Answer from the drawing. Dimensions are ordinates in mm from the lowest x, y and z of the part. A direction names the side the tool comes from. Give positions to 0.01 mm unless a question says otherwise; leave off trailing zeros. Loops run counter-clockwise (first coordinate to the right, second up) from the corner with the lowest first, then second, coordinate; pieces in that order, holes last.
Item 1: Section D-D, the plane x = 18 is taken. Give the vertices of the cut face in (y, z), and give its area (3 significant figures).
Item 2: Each of these flat-tipped pins is pushed along its axis until it touches: pin 1 Ø2 at (y, z) = (20.5, 26.5) entering from +X; pin 2 Ø10 at (x, y) = (26.5, 36) entering from +Z. Where does it stop, or does it pass through?
Item 3: A tool of negligible diameter and unlimited length cuts with its end or side. For the marked faces 1, 2 and 3, from which of +Z, -Z, +X, -X, +Y, -Y can it reach the whole face along a straight path? Write none if from no direction.
Item 4: Section B-B, the plane y = 41 is taken. Give the vertices of the cut face in (x, z).
Item 5: Consider line 1 along Y through (x, z) = (4, 37); line 2 along X through (y, z) = (17, 11); line 3 along Y through (x, z) = (65, 37). Determine where each line is inside the solid, lowest interval first.
Item 6: Section A-A, the plane z = 37 is taken. Give the vertices of the cut face in (x, y).
Item 7: The mould has two halves that part along X. Classify the marked faces 4, 5 and 6: pulls with the +X half, pulls with the -X half, needs draft (parallel to the pull), parting line crosses it, or undercut.
Item 8: Section C-C, the plane y = 26.5 is taken. Give the vertices of the cut face in (x, z), and give its area (3 significant figures).
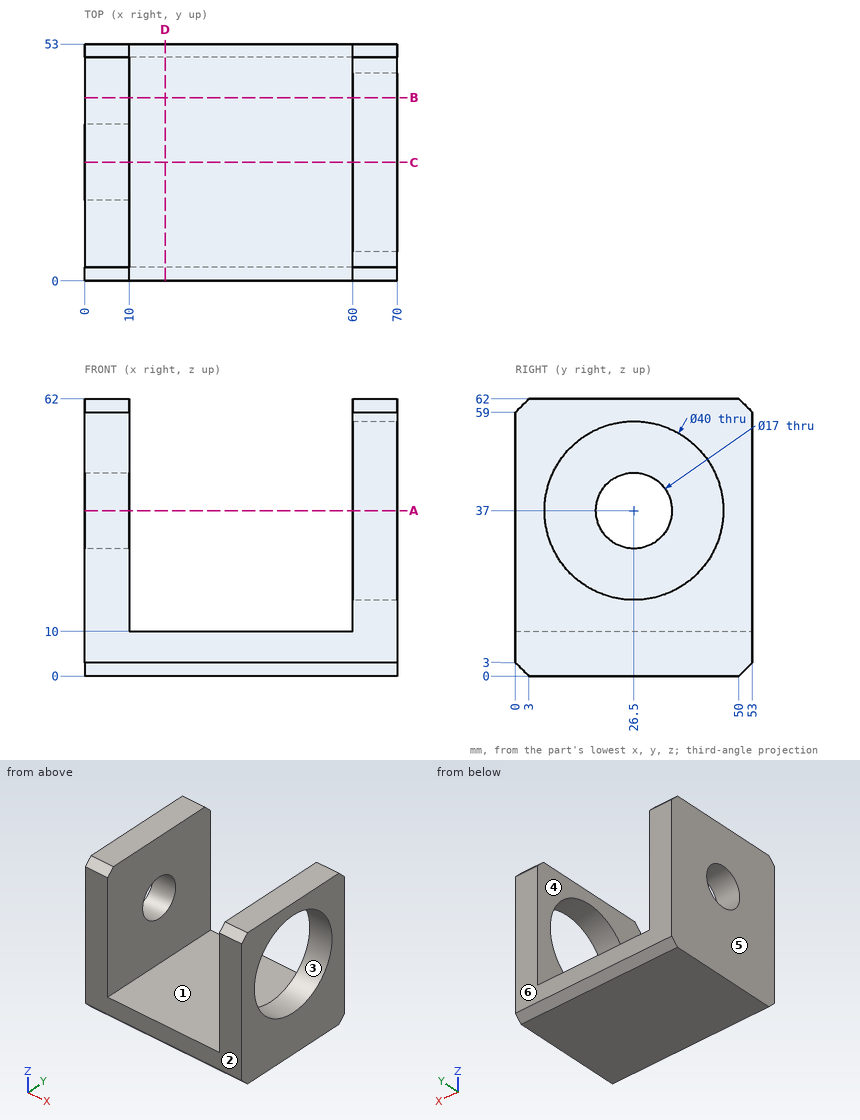
Worked answers:
1. outline: (0, 3) - (3, 0) - (50, 0) - (53, 3) - (53, 10) - (0, 10) - close
1. area: 521 mm2
2. pin 1: stops at x = 10
2. pin 2: stops at z = 10
3. face 1: +Z, +Y, -Y
3. face 2: +Z, -Z, +X, -X, -Y
3. face 3: +X
4. outline: (0, 0) - (70, 0) - (70, 23.23) - (60, 23.23) - (60, 10) - (10, 10) - (10, 62) - (0, 62) - close; (60, 50.77) - (70, 50.77) - (70, 62) - (60, 62) - close
5. line 1: y = 0 to 18, 35 to 53
5. line 2: x = 0 to 10, 60 to 70
5. line 3: y = 0 to 6.5, 46.5 to 53
6. outline: (0, 0) - (10, 0) - (10, 18) - (0, 18) - close; (0, 35) - (10, 35) - (10, 53) - (0, 53) - close; (60, 0) - (70, 0) - (70, 6.5) - (60, 6.5) - close; (60, 46.5) - (70, 46.5) - (70, 53) - (60, 53) - close
7. face 4: undercut
7. face 5: pulls with the -X half
7. face 6: needs draft
8. outline: (0, 0) - (70, 0) - (70, 17) - (60, 17) - (60, 10) - (10, 10) - (10, 28.5) - (0, 28.5) - close; (0, 45.5) - (10, 45.5) - (10, 62) - (0, 62) - close; (60, 57) - (70, 57) - (70, 62) - (60, 62) - close
8. area: 1,170 mm2
